For this review, take the finished solid that the model builds, in its own axes (mm). Coordinates: 2 decimals unless noted, no trailing zeros. Write each loop counter-clockwise with the first axis right and the second up, starting at its lowest first coordinate (ties: lowest second). Pieces come first, ordered by that corner, then holes. Notation, with made-up numbers: (70.25, 37) -> (76.25, 37) arc R21 cw to (76.25, 50) -> close; hole circle Ø4 at (52.5, 60.25). An arc over 180 degrees is marked (long way). One line per item, written item: value. Start each with the question number.
1) Add section B-B (z = 2). State the section outline as (x, y) points, and give its area (3 significant figures).
2) Add section A-A (x = -60). State the section outline as (y, z) points, and give its area (3 significant figures).
3) For probe 1 along Y at (x, z) = (47, 1.7); probe 2 along X at (y, z) = (27, 2.3); probe 3 along X at (y, z) = (-2, 3), list the stretches that pass through material, from the lowest coordinate up. Write a range as from..to.
4) Add section D-D (y = 0). State the section outline as (x, z) points.
5) For pin 1 Ø7.5 at (x, y) = (-8, 0) entering from -Z; pin 2 Ø6 at (x, y) = (52, 0) entering from -Z, all flat-tipped, find the tip position at first contact; note any pin that passes through.
6) Add section C-C (x = 52). State the section outline as (y, z) points.
7) Mouldability with a two-part tool opening along Y and no side actions: class faces 1 (the cylindrical face through (-77.15, -28.99, 2.03)), 2 (the cylindrical face through (-61.34, 27.11, 1.97)), 3 (the flat face through (-80, 0, 2)) as released by +Y, released by -Y, zero draft, split by the parting line, or undercut.
from build123d import *

# Parameters (mm, degrees)
SKETCH_1_W               = 160
SKETCH_1_H               = 64
EXTRUDE_1_DEPTH          = 4
FILLET_1_R               = 10
HOLE_WIZARD_M6_1_D       = 5
HOLE_WIZARD_2_AT_2_COUNT = 2
HOLE_WIZARD_2_AT_2_PITCH = 60


with BuildPart() as part:
    # 草图1 → 凸台-拉伸1 (new body)
    with BuildSketch(Plane.XY):
        Rectangle(SKETCH_1_W, SKETCH_1_H)
    extrude(amount=EXTRUDE_1_DEPTH)

    # 圆角1
    fillet_1_edges = [part.edges().sort_by_distance(p)[0] for p in [
        (80, -32, 2),
        (-80, -32, 2),
        (-80, 32, 2),
        (80, 32, 2),
    ]]
    fillet(fillet_1_edges, radius=FILLET_1_R)

    # M6 螺纹孔1 (through all)
    with Locations(Plane.XY.offset(4)):
        with Locations((-60, 25), (-60, -25), (47, 25), (47, -25)):
            Hole(HOLE_WIZARD_M6_1_D / 2)

    # 草图6 → 打孔尺寸(%根据)内六角花形半沉头螺钉的类型2 (revolve, cut)
    with BuildSketch(Plane.YZ.offset(52)):
        Polygon((0, 0), (0, 4), (3.3, 4), (3.3, 3.1), (6.4, 0), align=None)
    hole_wizard_2 = revolve(axis=Axis((52, 0, -6.35), (0, 0, 1)), mode=Mode.SUBTRACT)

    # 打孔尺寸(%根据)内六角花形半沉头螺钉的类型2 at 2: 打孔尺寸(%根据)内六角花形半沉头螺钉的类型2 ×2
    with Locations(*[(-i * HOLE_WIZARD_2_AT_2_PITCH, 0, 0) for i in range(1, HOLE_WIZARD_2_AT_2_COUNT)]):
        add(hole_wizard_2, mode=Mode.SUBTRACT)


solid = part.part
Numbers:
1. outline: (-80, -22) arc R10 ccw to (-70, -32) -> (70, -32) arc R10 ccw to (80, -22) -> (80, 22) arc R10 ccw to (70, 32) -> (-70, 32) arc R10 ccw to (-80, 22) -> close; hole circle Ø5 at (-60, -25); hole circle Ø5 at (-60, 25); hole circle Ø8.8 at (-8, 0); hole circle Ø5 at (47, -25); hole circle Ø5 at (47, 25); hole circle Ø8.8 at (52, 0)
1. area: 9,950 mm²
2. outline: (-32, 0) -> (-27.5, 0) -> (-27.5, 4) -> (-32, 4) -> close; (-22.5, 0) -> (22.5, 0) -> (22.5, 4) -> (-22.5, 4) -> close; (27.5, 0) -> (32, 0) -> (32, 4) -> (27.5, 4) -> close
2. area: 216 mm²
3. probe 1: -32..-27.5, -22.5..22.5, 27.5..32
3. probe 2: -78.66..-61.5, -58.5..45.5, 48.5..78.66
3. probe 3: -80..-10.75, -5.25..49.25, 54.75..80
4. outline: (-80, 0) -> (-14.4, 0) -> (-11.3, 3.1) -> (-11.3, 4) -> (-80, 4) -> close; (-4.7, 3.1) -> (-1.6, 0) -> (45.6, 0) -> (48.7, 3.1) -> (48.7, 4) -> (-4.7, 4) -> close; (55.3, 3.1) -> (58.4, 0) -> (80, 0) -> (80, 4) -> (55.3, 4) -> close
5. pin 1: z = 2.65
5. pin 2: through
6. outline: (-32, 0) -> (-6.4, 0) -> (-3.3, 3.1) -> (-3.3, 4) -> (-32, 4) -> close; (3.3, 3.1) -> (6.4, 0) -> (32, 0) -> (32, 4) -> (3.3, 4) -> close
7. face 1: released by -Y
7. face 2: undercut
7. face 3: zero draft
